```python
from build123d import *

# Parameters (mm, degrees)
SKETCH_11_R         = 3
SKETCH_11_R_2       = 2.5
F_0_GY_3030_1_DEPTH = 350


with BuildPart() as part:
    # 草图11 → 0国耀铝型材 GY-3030国标铝型材(1) (new body)
    with BuildSketch(Plane.YZ):
        with BuildLine():
            Line((-14, -15), (-3.15, -15))
            Line((-3.15, -15), (-3.15, -12.5))
            Line((-3.15, -12.5), (-5.15, -12.5))
            Line((-5.15, -12.5), (-5.15, -6.5))
            ThreePointArc((-5.15, -6.5), (-3.019390742, -5.122695475), (-0.555, -4.52))
            Line((-0.555, -4.52), (0, -4.2))
            Line((0, -4.2), (0.555, -4.52))
            ThreePointArc((0.555, -4.52), (3.019390742, -5.122695475), (5.15, -6.5))
            Line((5.15, -6.5), (5.15, -12.5))
            Line((5.15, -12.5), (3.15, -12.5))
            Line((3.15, -12.5), (3.15, -15))
            Line((3.15, -15), (14, -15))
            ThreePointArc((14, -15), (14.707106781, -14.707106781), (15, -14))
            Line((15, -14), (15, -3.15))
            Line((15, -3.15), (12.5, -3.15))
            Line((12.5, -3.15), (12.5, -5.15))
            Line((12.5, -5.15), (6.5, -5.15))
            ThreePointArc((6.5, -5.15), (5.12253592, -3.018923167), (4.52, -0.554))
            Line((4.52, -0.554), (4.2, 0))
            Line((4.2, 0), (4.52, 0.555))
            ThreePointArc((4.52, 0.555), (5.122695475, 3.019390742), (6.5, 5.15))
            Line((6.5, 5.15), (12.5, 5.15))
            Line((12.5, 5.15), (12.5, 3.15))
            Line((12.5, 3.15), (15, 3.15))
            Line((15, 3.15), (15, 14))
            ThreePointArc((15, 14), (14.707106781, 14.707106781), (14, 15))
            Line((14, 15), (3.15, 15))
            Line((3.15, 15), (3.15, 12.5))
            Line((3.15, 12.5), (5.15, 12.5))
            Line((5.15, 12.5), (5.15, 6.5))
            ThreePointArc((5.15, 6.5), (3.019292492, 5.123227892), (0.555, 4.521))
            Line((0.555, 4.521), (0, 4.2))
            Line((0, 4.2), (-0.555, 4.521))
            ThreePointArc((-0.555, 4.521), (-3.019292492, 5.123227892), (-5.15, 6.5))
            Line((-5.15, 6.5), (-5.15, 12.5))
            Line((-5.15, 12.5), (-3.15, 12.5))
            Line((-3.15, 12.5), (-3.15, 15))
            Line((-3.15, 15), (-14, 15))
            ThreePointArc((-14, 15), (-14.707106781, 14.707106781), (-15, 14))
            Line((-15, 14), (-15, 3.15))
            Line((-15, 3.15), (-12.5, 3.15))
            Line((-12.5, 3.15), (-12.5, 5.15))
            Line((-12.5, 5.15), (-6.5, 5.15))
            ThreePointArc((-6.5, 5.15), (-5.122695475, 3.019390742), (-4.52, 0.555))
            Line((-4.52, 0.555), (-4.2, 0))
            Line((-4.2, 0), (-4.52, -0.554))
            ThreePointArc((-4.52, -0.554), (-5.12253592, -3.018923167), (-6.5, -5.15))
            Line((-6.5, -5.15), (-12.5, -5.15))
            Line((-12.5, -5.15), (-12.5, -3.15))
            Line((-12.5, -3.15), (-15, -3.15))
            Line((-15, -3.15), (-15, -14))
            ThreePointArc((-15, -14), (-14.707106781, -14.707106781), (-14, -15))
        make_face()
        with Locations((9.8, 9.9)):
            Circle(SKETCH_11_R, mode=Mode.SUBTRACT)
        with Locations((9.8, -9.9)):
            Circle(SKETCH_11_R, mode=Mode.SUBTRACT)
        Circle(SKETCH_11_R_2, mode=Mode.SUBTRACT)
        with Locations((-9.8, 9.9)):
            Circle(SKETCH_11_R, mode=Mode.SUBTRACT)
        with Locations((-10, -9.9)):
            Circle(SKETCH_11_R, mode=Mode.SUBTRACT)
    extrude(amount=F_0_GY_3030_1_DEPTH)


solid = part.part
```
Source: CAD feature listing. Evaluate the final solid. Frame: model axes, mm. A direction names the side the tool comes from. Round coordinates to 2 decimals unless told otherwise and drop trailing zeros.
(1) Section query A-A (x = 85). Give the number of separate pieces and of enclosed holes in the cut face, and give its area (3 significant figures).
From the geometry:
separate pieces: 1
enclosed holes: 5
area: 399 mm2
(2) Access query for faces 4 (the flat face through (173, 8, -15)), 5 (the flat face through (173, -5.15, -10)). Directions: +Z, -Z, +X, -X, +Y, -Y. A direction counts if a zero-diameter tool reaches every point of the face in a straight line with its end or side. Return the directions, or none.
From the geometry:
face 4: -Z, +X, -X, +Y, -Y
face 5: +X, -X
(3) Pull-direction query (Y, two-part tool) for faces 1 (the flat face through (173, 9, 5.15)), 2 (the flat face through (173, -15, -8)), 3 (the flat face through (173, -9, -15)); classes: +Y half, -Y half, draft (parallel to the pull), parting line (faces both ways), or undercut.
From the geometry:
face 1: undercut
face 2: -Y half
face 3: draft
(4) Material intervals for probe 1 along Z at (x, y) = (151.5, -9.8); probe 2 along Z at (x, y) = (281.5, 8); probe 3 along Z at (x, y) = (112.5, 13), sorted ascending.
From the geometry:
probe 1: z = -15 to -12.89, -6.91 to -5.15, 5.15 to 6.9, 12.9 to 15
probe 2: z = -15 to -12.3, -7.5 to -5.15, 5.15 to 7.5, 12.3 to 15
probe 3: z = -15 to -3.15, 3.15 to 15
